from build123d import *

# Parameters (mm, degrees)
SKETCH1_W                                           = 8.5
SKETCH1_H                                           = 3.5
BOSS_EXTRUDE1_DEPTH                                 = 2.5
M3_TAPPED_HOLE1_D                                   = 2.5
HOLE_SIZE_BY_SOCKET_HEAD_CAP_SCREW_TYPE_D           = 3.4
HOLE_SIZE_BY_SOCKET_HEAD_CAP_SCREW_TYPE_CBORE_D     = 6
HOLE_SIZE_BY_SOCKET_HEAD_CAP_SCREW_TYPE_CBORE_DEPTH = 3.4
CHAMFER2_SIZE                                       = 5
CHAMFER3_SIZE                                       = 2


with BuildPart() as part:
    # Sketch1 → Boss-Extrude1 (new, symmetric)
    with BuildSketch(Plane.XY):
        Polygon((-12.5, 2), (-12.5, -5.5), (12.5, -5.5), (12.5, 2), (4, 2), (4, 5.5), (-4, 5.5), (-4, 2), align=None)
        with Locations((8.25, 3.75)):
            Rectangle(SKETCH1_W, SKETCH1_H)
        with Locations((-8.25, 3.75)):
            Rectangle(SKETCH1_W, SKETCH1_H)
    extrude(amount=BOSS_EXTRUDE1_DEPTH, both=True)

    # M3 Tapped Hole1 (through all)
    with Locations(Plane.XY.offset(2.5)):
        with Locations((-7.5, 2.5), (7.5, 2.5)):
            Hole(M3_TAPPED_HOLE1_D / 2)

    # Hole size (by socket head cap screw type)1 (through all)
    with Locations(Plane.XY.offset(2.5)):
        with Locations((9, -2.25), (-9, -2.25)):
            CounterBoreHole(HOLE_SIZE_BY_SOCKET_HEAD_CAP_SCREW_TYPE_D / 2, HOLE_SIZE_BY_SOCKET_HEAD_CAP_SCREW_TYPE_CBORE_D / 2, HOLE_SIZE_BY_SOCKET_HEAD_CAP_SCREW_TYPE_CBORE_DEPTH)

    # Chamfer2
    chamfer2_edges = [part.edges().sort_by_distance(p)[0] for p in [
        (12.5, 5.5, 0),
        (-12.5, 5.5, 0),
    ]]
    chamfer(chamfer2_edges, length=CHAMFER2_SIZE)

    # Chamfer3
    chamfer3_edges = [part.edges().sort_by_distance(p)[0] for p in [
        (12.5, -5.5, 0),
        (-12.5, -5.5, 0),
    ]]
    chamfer(chamfer3_edges, length=CHAMFER3_SIZE)


solid = part.part
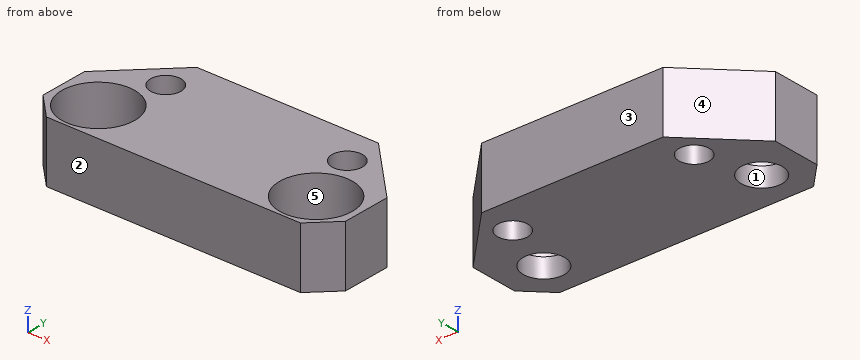
Read the model definition and answer for the solid it produces. Units are mm, in the model's axes. Face numbers are marked on the shaded views. A direction names the side the tool comes from. Round coordinates to 2 decimals unless told otherwise and drop trailing zeros. Write each loop counter-clockwise with the first axis right and the second up, starting at its lowest first coordinate (ties: lowest second). Pieces come first, ordered by that corner, then holes.
1. Straight lines are drawn through the part: L1, parallel to X at y = -1.5, z = -1; L2, parallel to X at y = -0.25, z = -0.1; L3, parallel to Y at x = -9, z = -1.35. For each, find the intervals that lie inside material, in ascending order.
2. Which of the six approach directions +Z, -Z, +X, -X, +Y, -Y give full straight-line access (tool end or side, diameter ignored) to the marked faces 4 and 5?
3. The part is cut by section B-B, the plane z = -1.8. Determine the outline of the cut face in (x, y), then the cut area to 3 significant figures.
4. The part is cut by section D-D, the plane x = 9. Determine the outline of the cut face in (y, z).
5. Given pin 1 Ø1.8 at (x, y) = (9, -3) entering from +Z; pin 2 Ø5.5 at (x, y) = (-9, -2.25) entering from +Z, each flat-ended and moving along its own axis, determine where each tip first touches the part or whether it passes through.
6. Determine the mould class of the marked faces 1, 2 and 3 for opening direction Y: pulls with the +Y half, pulls with the -Y half, needs draft (parallel to the pull), parting line crosses it, or undercut.
7. The part is cut by section A-A, the plane y = 2.5. Determine the outline of the cut face in (x, z).
8. The part is cut by section C-C, the plane x = -8. Determine the outline of the cut face in (y, z), then the cut area to 3 significant figures.
Values:
1. L1: x = -12.5 to -10.53, -7.47 to 7.47, 10.53 to 12.5
1. L2: x = -12.5 to -11.24, -6.76 to 6.76, 11.24 to 12.5
1. L3: y = -5.5 to -3.95, -0.55 to 4
2. face 4: +Z, -Z, -X, +Y
2. face 5: +Z
3. outline: (-12.5, -3.5) - (-10.5, -5.5) - (10.5, -5.5) - (12.5, -3.5) - (12.5, 0.5) - (7.5, 5.5) - (-7.5, 5.5) - (-12.5, 0.5) - close; hole circle Ø3.4 at (-9, -2.25); hole circle Ø2.5 at (-7.5, 2.5); hole circle Ø2.5 at (7.5, 2.5); hole circle Ø3.4 at (9, -2.25)
3. area: 218 mm2
4. outline: (-5.5, -2.5) - (-3.95, -2.5) - (-3.95, -0.9) - (-5.25, -0.9) - (-5.25, 2.5) - (-5.5, 2.5) - close; (-0.55, -2.5) - (4, -2.5) - (4, 2.5) - (0.75, 2.5) - (0.75, -0.9) - (-0.55, -0.9) - close
5. pin 1: passes through
5. pin 2: stops at z = -0.9
6. face 1: undercut
6. face 2: pulls with the -Y half
6. face 3: pulls with the +Y half
7. outline: (-10.5, -2.5) - (-8.75, -2.5) - (-8.75, 2.5) - (-10.5, 2.5) - close; (-6.25, -2.5) - (6.25, -2.5) - (6.25, 2.5) - (-6.25, 2.5) - close; (8.75, -2.5) - (10.5, -2.5) - (10.5, 2.5) - (8.75, 2.5) - close
8. outline: (-5.5, -2.5) - (-3.62, -2.5) - (-3.62, -0.9) - (-5.08, -0.9) - (-5.08, 2.5) - (-5.5, 2.5) - close; (-0.88, -2.5) - (1.35, -2.5) - (1.35, 2.5) - (0.58, 2.5) - (0.58, -0.9) - (-0.88, -0.9) - close; (3.65, -2.5) - (5, -2.5) - (5, 2.5) - (3.65, 2.5) - close
8. area: 17.4 mm2
